Read the model definition and answer for the solid it produces. Units are mm, in the model's axes. Coordinates: 2 decimals unless noted, no trailing zeros. Loops run counter-clockwise (first coordinate to the right, second up) from the corner with the lowest first, then second, coordinate; pieces in that order, holes last. Notation, with made-up numbers: (36.5, -39.75) -> (60.5, -39.75) arc R7 cw to (60.5, -35.75) -> close; hole circle Ø4 at (45.5, -10.5). An arc over 180 degrees is marked (long way). Answer as a JSON object with one key per item and string values. Group by question number.
1) Determine the mould class of faces 1 (the face through (49, 37, 2)), 2 (the face through (49, 19, 5)), 3 (the face through (97.08, 24.14, 2.54)) for opening direction Y: released by +Y, released by -Y, zero draft, split by the parting line, or undercut.
2) Section B-B, the plane x = 5 is taken. Give the vertices of the cut face in (y, z), plus the area to 4 significant figures.
3) Consider probe 1 along Y at (x, z) = (5, 3.95). Determine where the line is inside the solid, lowest interval first. Write a range as [from, to].
4) Section A-A, the plane y = 25 is taken. Give the vertices of the cut face in (x, z).
from build123d import *

# Parameters (mm, degrees)
SKETCH_1_W          = 100
SKETCH_1_H          = 37
EXTRUDE_1_DEPTH     = 5
SKETCH_2_R          = 2.25
CUT_EXTRUDE_1_DEPTH = 5


with BuildPart() as part:
    # 草图1 → 凸台-拉伸1 (new body)
    with BuildSketch(Plane.XY):
        with Locations((50, 18.5)):
            Rectangle(SKETCH_1_W, SKETCH_1_H)
    extrude(amount=EXTRUDE_1_DEPTH)

    # 草图2 → 切除-拉伸1 (cut)
    with BuildSketch(Plane.XY.offset(5)):
        with Locations((5, 25)):
            Circle(SKETCH_2_R)
        with Locations((95, 25)):
            Circle(SKETCH_2_R)
    extrude(amount=-CUT_EXTRUDE_1_DEPTH, mode=Mode.SUBTRACT)


solid = part.part
Determined:
{
 "1": {"face 1": "released by +Y", "face 2": "zero draft", "face 3": "undercut"},
 "2": {"outline": "(0, 0) -> (22.75, 0) -> (22.75, 5) -> (0, 5) -> close; (27.25, 0) -> (37, 0) -> (37, 5) -> (27.25, 5) -> close", "area": "162.5 mm²"},
 "3": {"probe 1": "[0, 22.75], [27.25, 37]"},
 "4": {"outline": "(0, 0) -> (2.75, 0) -> (2.75, 5) -> (0, 5) -> close; (7.25, 0) -> (92.75, 0) -> (92.75, 5) -> (7.25, 5) -> close; (97.25, 0) -> (100, 0) -> (100, 5) -> (97.25, 5) -> close"}
}
